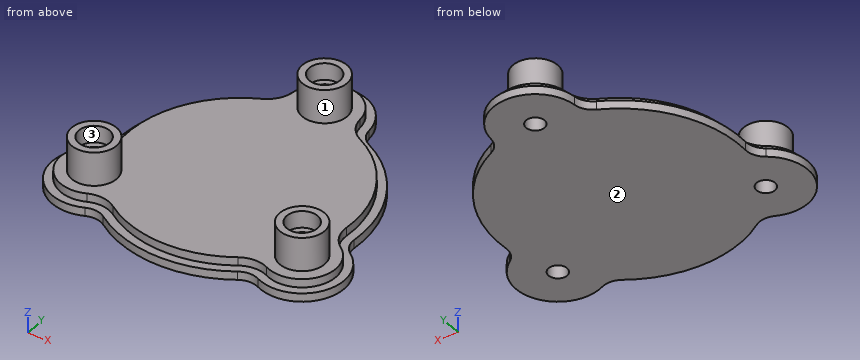
```python
from build123d import *

# Parameters (mm, degrees)
BASE_PLATE_3MM_DEPTH              = 3
RAISED_STEP_3MM_DEPTH             = 3
BOSS_PROFILE_3X_16_R              = 8
BOSSES_3X_16X12_DEPTH             = 12
COUNTERBORE_PROFILE_3X_11_R       = 5.5
COUNTERBORES_3X_11X6_DEPTH        = 6
CLEARANCE_HOLE_PROFILE_3X_6_6_R   = 3.3
CLEARANCE_HOLES_3X_6_6_THRU_DEPTH = 146


with BuildPart() as part:
    # Base Plate Profile → Base Plate 3mm (new body)
    with BuildSketch(Plane.XY):
        with BuildLine():
            ThreePointArc((-18.846153454, 38.65), (-37.239092363, 21.5), (-42.894958583, -3.003752345))
            ThreePointArc((-42.894958583, -3.003752345), (-43.557934635, -6.502479184), (-45.856433127, -9.222319513))
            ThreePointArc((-45.856433127, -9.222319513), (-50.229473419, -29), (-30.914979544, -35.101676259))
            ThreePointArc((-30.914979544, -35.101676259), (-27.410279478, -34.471038339), (-24.048805129, -35.646247655))
            ThreePointArc((-24.048805129, -35.646247655), (0, -43), (24.048805129, -35.646247655))
            ThreePointArc((24.048805129, -35.646247655), (27.410279478, -34.471038339), (30.914979544, -35.101676259))
            ThreePointArc((30.914979544, -35.101676259), (50.22947342, -29), (45.856433127, -9.222319513))
            ThreePointArc((45.856433127, -9.222319513), (43.557934635, -6.502479184), (42.894958583, -3.003752345))
            ThreePointArc((42.894958583, -3.003752345), (37.239092363, 21.5), (18.846153454, 38.65))
            ThreePointArc((18.846153454, 38.65), (16.147655157, 40.973517522), (14.941453584, 44.323995772))
            ThreePointArc((14.941453584, 44.323995772), (0, 58), (-14.941453584, 44.323995772))
            ThreePointArc((-14.941453584, 44.323995772), (-16.147655157, 40.973517522), (-18.846153454, 38.65))
        make_face()
    extrude(amount=BASE_PLATE_3MM_DEPTH)

    # Raised Step Profile → Raised Step 3mm (add)
    with BuildSketch(Plane.XY.offset(3)):
        with BuildLine():
            ThreePointArc((-17.531305538, 35.953488372), (-13.676307972, 39.272799119), (-11.953162867, 44.059196617))
            ThreePointArc((-11.953162867, 44.059196617), (0, 55), (11.953162867, 44.059196617))
            ThreePointArc((11.953162867, 44.059196617), (13.676307972, 39.272799119), (17.531305538, 35.953488372))
            ThreePointArc((17.531305538, 35.953488372), (34.641016151, 20), (39.902287054, -2.794188228))
            ThreePointArc((39.902287054, -2.794188228), (40.8493957, -7.792369426), (44.132964974, -11.67785561))
            ThreePointArc((44.132964974, -11.67785561), (47.631397208, -27.5), (32.179802107, -32.381341007))
            ThreePointArc((32.179802107, -32.381341007), (27.173087728, -31.480429693), (22.370981516, -33.159300144))
            ThreePointArc((22.370981516, -33.159300144), (0, -40), (-22.370981516, -33.159300144))
            ThreePointArc((-22.370981516, -33.159300144), (-27.173087728, -31.480429693), (-32.179802107, -32.381341007))
            ThreePointArc((-32.179802107, -32.381341007), (-47.631397208, -27.5), (-44.132964974, -11.67785561))
            ThreePointArc((-44.132964974, -11.67785561), (-40.8493957, -7.792369426), (-39.902287054, -2.794188228))
            ThreePointArc((-39.902287054, -2.794188228), (-34.641016151, 20), (-17.531305538, 35.953488372))
        make_face()
    extrude(amount=RAISED_STEP_3MM_DEPTH)

    # Boss Profile 3xØ16 → Bosses 3xØ16x12 (add)
    with BuildSketch(Plane.XY.offset(6)):
        with Locations((0, 43)):
            Circle(BOSS_PROFILE_3X_16_R)
        with Locations((37.239092363, -21.5)):
            Circle(BOSS_PROFILE_3X_16_R)
        with Locations((-37.239092363, -21.5)):
            Circle(BOSS_PROFILE_3X_16_R)
    extrude(amount=BOSSES_3X_16X12_DEPTH)

    # Counterbore Profile 3xØ11 → Counterbores 3xØ11x6 (cut)
    with BuildSketch(Plane.XY.offset(18)):
        with Locations((0, 43)):
            Circle(COUNTERBORE_PROFILE_3X_11_R)
        with Locations((37.239092363, -21.5)):
            Circle(COUNTERBORE_PROFILE_3X_11_R)
        with Locations((-37.239092363, -21.5)):
            Circle(COUNTERBORE_PROFILE_3X_11_R)
    extrude(amount=-COUNTERBORES_3X_11X6_DEPTH, mode=Mode.SUBTRACT)

    # Clearance Hole Profile 3xØ6.6 → Clearance Holes 3xØ6.6 Thru (cut)
    with BuildSketch(Plane.XY.offset(12)):
        with Locations((0, 43)):
            Circle(CLEARANCE_HOLE_PROFILE_3X_6_6_R)
        with Locations((37.239092363, -21.5)):
            Circle(CLEARANCE_HOLE_PROFILE_3X_6_6_R)
        with Locations((-37.239092363, -21.5)):
            Circle(CLEARANCE_HOLE_PROFILE_3X_6_6_R)
    extrude(amount=-CLEARANCE_HOLES_3X_6_6_THRU_DEPTH, mode=Mode.SUBTRACT)


solid = part.part
```
Build history of the part. All positions in model axes, mm. Face numbers are marked on the shaded views. Round coordinates to 2 decimals unless told otherwise and drop trailing zeros. Loops run counter-clockwise (first coordinate to the right, second up) from the corner with the lowest first, then second, coordinate; pieces in that order, holes last.
Item 1: Saw through at D-D (z = 14.5). List the corners of the cut face in (x, y), then the cut area to 3 significant figures.
Item 2: Two-plate mould, pull along X, no slides. Class the marked faces 1, 2 and 3: released by +X, released by -X, zero draft, split by the parting line, or undercut.
Item 3: Saw through at B-B (y = -21.5). State how many separate pieces and enclosed holes the cut face has, then the cut area to 3 significant figures.
Item 4: Drill centre lines: line 1 along X through (y, z) = (43.5, 14.25); line 2 along Y through (x, z) = (0, 1.75); line 3 along Z through (x, y) = (34, -0.5). Where is each one in solid material? Low to high.
Item 5: Saw through at C-C (x = 0). List the corners of the cut face in (y, z).
Item 6: Saw through at A-A (z = 8.25). List the corners of the cut face in (x, y), then the cut area to 3 significant figures.
Item 7: Pin check, flat tips, straight feed: P1, Ø3.5, axis at x = 36, y = -23, coming from the +Z side; P2, Ø1, axis at y = 6, z = 5.5, coming from the -X side; P3, Ø3, axis at y = 36.5, z = 8, coming from the -X side (3 decimals). Stop position of each tip, or through.
Worked answers:
1. outline: circle Ø16 at (-37.24, -21.5); circle Ø16 at (0, 43); circle Ø16 at (37.24, -21.5); hole circle Ø11 at (-37.24, -21.5); hole circle Ø11 at (0, 43); hole circle Ø11 at (37.24, -21.5)
1. area: 318 mm2
2. face 1: split by the parting line
2. face 2: zero draft
2. face 3: undercut
3. separate pieces: 3
3. enclosed holes: 0
3. area: 702 mm2
4. line 1: x = -7.98 to -5.48, 5.48 to 7.98
4. line 2: y = -43 to 39.7, 46.3 to 58
4. line 3: z = 0 to 6
5. outline: (-43, 0) - (39.7, 0) - (39.7, 12) - (37.5, 12) - (37.5, 18) - (35, 18) - (35, 6) - (-40, 6) - (-40, 3) - (-43, 3) - close; (46.3, 0) - (58, 0) - (58, 3) - (55, 3) - (55, 6) - (51, 6) - (51, 18) - (48.5, 18) - (48.5, 12) - (46.3, 12) - close
6. outline: circle Ø16 at (-37.24, -21.5); circle Ø16 at (0, 43); circle Ø16 at (37.24, -21.5); hole circle Ø6.6 at (-37.24, -21.5); hole circle Ø6.6 at (0, 43); hole circle Ø6.6 at (37.24, -21.5)
6. area: 501 mm2
7. P1: stops at z = 12
7. P2: stops at x = -39.62
7. P3: stops at x = -6.245
